from build123d import *

# Parameters (mm, degrees)
EXTRUDE_1_DEPTH        = 21
SKETCH_2_R             = 5.5
CUT_EXTRUDE_1_DEPTH    = 9
SKETCH_3_R             = 3.5
CUT_EXTRUDE_2_DEPTH    = 69.483574673
HOLE_WIZARD_M6_1_D     = 5
HOLE_WIZARD_M6_1_DEPTH = 17
HOLE_WIZARD_M6_1_TIP   = 1.502151548


with BuildPart() as part:
    # 草图1 → 凸台-拉伸1 (new body)
    with BuildSketch(Plane.XY):
        Polygon((0, 20), (20, 0), (35.5, 0), (39, 3.5), (39, 19), (29, 55), (3.5, 55), (0, 51.5), align=None)
    extrude(amount=EXTRUDE_1_DEPTH)

    # 草图2 → 切除-拉伸1 (cut)
    with BuildSketch(Plane.XY.offset(21)):
        with Locations((16.5, 47)):
            Circle(SKETCH_2_R)
        with Locations((16.5, 16)):
            Circle(SKETCH_2_R)
    extrude(amount=-CUT_EXTRUDE_1_DEPTH, mode=Mode.SUBTRACT)

    # 草图3 → 切除-拉伸2 (cut, through all)
    with BuildSketch(Plane.XY.offset(12)):
        with Locations((16.5, 47)):
            Circle(SKETCH_3_R)
        with Locations((16.5, 16)):
            Circle(SKETCH_3_R)
    extrude(amount=-CUT_EXTRUDE_2_DEPTH, mode=Mode.SUBTRACT)

    # M6 螺纹孔1
    with Locations(Plane(origin=(17.5, 32, 21), x_dir=(1, 0, 0), z_dir=(0, 0, 1))):
        with Locations((0, 0), (14.112362721, -14.171845978)):
            Hole(HOLE_WIZARD_M6_1_D / 2, depth=HOLE_WIZARD_M6_1_DEPTH)
            with Locations((0, 0, -(HOLE_WIZARD_M6_1_DEPTH + HOLE_WIZARD_M6_1_TIP / 2))):  # 118° drill point
                Cone(0, HOLE_WIZARD_M6_1_D / 2, HOLE_WIZARD_M6_1_TIP, mode=Mode.SUBTRACT)


solid = part.part
The model under review builds one solid part; all positions refer to its coordinate system, in mm. A direction names the side the tool comes from. Give positions to 0.01 mm unless a question says otherwise; leave off trailing zeros. Order: outer loops, then holes, each group sorted by start corner. A loop starts at its lowest first (then second) coordinate and runs counter-clockwise, first axis right, second up. Notation, with made-up numbers: M 54.5,65 L 95.5,65 A19 ccw 95.5,100 Z; hole C 83,-32.5 d9. An arc over 180 degrees is marked long. Answer in a Markdown table with one row per item. Add a question column.
1. Machinability: for faces 1 (the flat face through (16, 12, 12)), 2 (the flat face through (1.8, 53.3, 10.4)), which of the approach directions +Z, -Z, +X, -X, +Y, -Y give a long, thin tool a straight path to every point of the face, cutting with its end or side? Answer none if there is none.
2. Mouldability with a two-part tool opening along X and no side actions: class faces 3 (the flat face through (28, 0, 10)), 4 (the flat face through (34, 37, 10)), 5 (the flat face through (16, 43, 12)), 6 (the cylindrical face through (15.784, 52.453, 16.563)) as released by +X, released by -X, zero draft, split by the parting line, or undercut.
3. For pin 1 Ø4 at (y, z) = (46, 7) entering from +X; pin 2 Ø4 at (x, y) = (16.5, 47) entering from -Z; pin 3 Ø8 at (x, y) = (16.5, 16) entering from +Z; pin 4 Ø5 at (y, z) = (11, 5) entering from -X, all flat-tipped, find the tip position at first contact; note any pin that passes through.
4. Add section A-A on y = 47. State the section outline as (x, z) points.
5. Add section D-D on x = 16.5. Count the separate pieces of the cut face and the enclosed holes in it, plus the area to 3 significant figures.
6. To check wall thickness, follow line 1 along Y through (x, z) = (16.5, 8.25); line 2 along Y through (x, z) = (11.5, 13.75); line 3 along Y through (x, z) = (16.5, 18.75). State the ranges of each line that lie inside material, in increasing order.
7. Add section B-B on z = 19.25. State the section outline as (x, y) points.
8. Add section C-C on x = 6.5. State the section outline as (y, z) points, plus the area to 4 significant figures.
The answers:
| question | item | result |
|---|---|---|
| 1 | face 1 | +Z |
| 1 | face 2 | +Z, -Z, -X, +Y |
| 2 | face 3 | zero draft |
| 2 | face 4 | released by +X |
| 2 | face 5 | undercut |
| 2 | face 6 | undercut |
| 3 | pin 1 | x = 32.06 |
| 3 | pin 2 | through |
| 3 | pin 3 | z = 12 |
| 3 | pin 4 | x = 6.5 |
| 4 | outline | M 0,0 L 13,0 L 13,12 L 11,12 L 11,21 L 0,21 Z; M 20,0 L 31.22,0 L 31.22,21 L 22,21 L 22,12 L 20,12 Z |
| 5 | separate pieces | 3 |
| 5 | enclosed holes | 0 |
| 5 | area | 635 mm2 |
| 6 | line 1 | 3.5 to 12.5, 19.5 to 29.71, 34.29 to 43.5, 50.5 to 55 |
| 6 | line 2 | 8.5 to 13.71, 18.29 to 44.71, 49.29 to 55 |
| 6 | line 3 | 3.5 to 10.5, 21.5 to 29.71, 34.29 to 41.5, 52.5 to 55 |
| 7 | outline | M 0,20 L 20,0 L 35.5,0 L 39,3.5 L 39,19 L 29,55 L 3.5,55 L 0,51.5 Z; hole C 16.5,16 d11; hole C 16.5,47 d11; hole C 17.5,32 d5; hole C 31.61,17.83 d5 |
| 8 | outline | M 13.5,0 L 55,0 L 55,21 L 13.5,21 Z |
| 8 | area | 871.5 mm2 |
